Can you work these out from the model? Positions are in its coordinate system, mm. A direction names the side the tool comes from. Give positions to 0.01 mm unless a question says otherwise; leave off trailing zeros. Loops run counter-clockwise (first coordinate to the right, second up) from the corner with the lowest first, then second, coordinate; pieces in that order, holes last. Notation, with made-up numbers: M -5,83 L 20,83 A17 ccw 20,88 Z; hole C 70.5,59 d4. An arc over 180 degrees is marked long. Use CSV: the item, a comma, the result in double quotes.
from build123d import *

# Parameters (mm, degrees)
SKETCH1_R                 = 15
BOSS_EXTRUDE1_DEPTH       = 52
SKETCH2_R                 = 17.5
BOSS_EXTRUDE2_DEPTH       = 43
SKETCH3_R                 = 22.5
BOSS_EXTRUDE3_DEPTH       = 12
SKETCH4_R                 = 15
BOSS_EXTRUDE4_DEPTH       = 40
SKETCH5_R                 = 13.5
BOSS_EXTRUDE5_DEPTH       = 43
SKETCH6_R                 = 12.5
BOSS_EXTRUDE6_DEPTH       = 28
CHAMFER1_SIZE             = 1
CHAMFER2_SIZE             = 1
CHAMFER3_SIZE             = 0.5
CUT_EXTRUDE1_START        = 12.5
CUT_EXTRUDE1_DEPTH        = 20
CUT_EXTRUDE2_START        = 8.5
CUT_EXTRUDE2_DEPTH        = 10
M8X1_0_TAPPED_HOLE1_D     = 7
M8X1_0_TAPPED_HOLE1_DEPTH = 19
M8X1_0_TAPPED_HOLE1_TIP   = 2.103012167


with BuildPart() as part:
    # Sketch1 → Boss-Extrude1 (new body)
    with BuildSketch(Plane.XY):
        with Locations(Location((0, 0, 0), (0, 0, 180))):
            Circle(SKETCH1_R)
    extrude(amount=BOSS_EXTRUDE1_DEPTH)

    # Sketch2 → Boss-Extrude2 (add)
    with BuildSketch(Plane.XY.offset(52)):
        Circle(SKETCH2_R)
    extrude(amount=BOSS_EXTRUDE2_DEPTH)

    # Sketch3 → Boss-Extrude3 (add)
    with BuildSketch(Plane.XY.offset(95)):
        Circle(SKETCH3_R)
    extrude(amount=BOSS_EXTRUDE3_DEPTH)

    # Sketch4 → Boss-Extrude4 (add)
    with BuildSketch(Plane.XY.offset(107)):
        with Locations(Location((0, 0, 0), (0, 0, 180))):
            Circle(SKETCH4_R)
    extrude(amount=BOSS_EXTRUDE4_DEPTH)

    # Sketch5 → Boss-Extrude5 (add)
    with BuildSketch(Plane.XY.offset(147)):
        Circle(SKETCH5_R)
    extrude(amount=BOSS_EXTRUDE5_DEPTH)

    # Sketch6 → Boss-Extrude6 (add)
    with BuildSketch(Plane.XY.offset(190)):
        Circle(SKETCH6_R)
    extrude(amount=BOSS_EXTRUDE6_DEPTH)

    # Chamfer1
    chamfer1_edges = [part.edges().sort_by_distance(p)[0] for p in [
        (15, 0, 0),
    ]]
    chamfer(chamfer1_edges, length=CHAMFER1_SIZE)

    # Chamfer2
    chamfer2_edges = [part.edges().sort_by_distance(p)[0] for p in [
        (15, 0, 147),
        (-12.5, 0, 218),
        (-17.5, 0, 52),
    ]]
    chamfer(chamfer2_edges, length=CHAMFER2_SIZE)

    # Chamfer3
    chamfer3_edges = [part.edges().sort_by_distance(p)[0] for p in [
        (-22.5, 0, 95),
        (-22.5, 0, 107),
    ]]
    chamfer(chamfer3_edges, length=CHAMFER3_SIZE)

    # Sketch7 → Cut-Extrude1 (cut)
    with BuildSketch(Plane(origin=(0, 0, 0), x_dir=(1, 0, 0), z_dir=(0, 1, 0)).offset(CUT_EXTRUDE1_START)):
        with BuildLine():
            Line((5, -67), (5, -82))
            ThreePointArc((5, -82), (0, -87), (-5, -82))
            Line((-5, -82), (-5, -67))
            ThreePointArc((-5, -67), (0, -62), (5, -67))
        make_face()
    extrude(amount=CUT_EXTRUDE1_DEPTH, mode=Mode.SUBTRACT)

    # Sketch8 → Cut-Extrude2 (cut)
    with BuildSketch(Plane(origin=(0, 0, 0), x_dir=(1, 0, 0), z_dir=(0, 1, 0)).offset(CUT_EXTRUDE2_START)):
        with BuildLine():
            Line((4, -198), (4, -210))
            ThreePointArc((4, -210), (0, -214), (-4, -210))
            Line((-4, -210), (-4, -198))
            ThreePointArc((-4, -198), (0, -194), (4, -198))
        make_face()
    extrude(amount=CUT_EXTRUDE2_DEPTH, mode=Mode.SUBTRACT)

    # M8x1.0 Tapped Hole1
    with Locations(Plane.XY.offset(218)):
        with Locations((0, 0)):
            Hole(M8X1_0_TAPPED_HOLE1_D / 2, depth=M8X1_0_TAPPED_HOLE1_DEPTH)
            with Locations((0, 0, -(M8X1_0_TAPPED_HOLE1_DEPTH + M8X1_0_TAPPED_HOLE1_TIP / 2))):  # 118° drill point
                Cone(0, M8X1_0_TAPPED_HOLE1_D / 2, M8X1_0_TAPPED_HOLE1_TIP, mode=Mode.SUBTRACT)


solid = part.part
Q1. If we mould it in two halves opening along Z, with no side actions, what happens to faces 4 (the cylindrical face through (-8.06, -12.65, 26.14)), 5 (the cylindrical face through (0, 15, 87)), 6 (the flat face through (5, 15, 74)), 7 (the flat face through (14.4, 5.2, 107))? For each: released by +Z, released by -Z, zero draft, split by the parting line, or undercut.
Model answer:
face 4,"zero draft"
face 5,"undercut"
face 6,"undercut"
face 7,"released by +Z"
Q2. I want a section at A-A, the plane z = 47. Please give me the cut outline in (x, y).
Model answer:
outline,"C 0,0 d30"
Q3. Please list where these lines run through material, in increasing order: L1, parallel to Y at x = 0, z = 211.5; L2, parallel to X at y = 1, z = 204; L3, parallel to Z at x = 4, y = 14.5. Write a range as from..to.
Model answer:
L1,"-12.5..-3.5, 3.5..8.5"
L2,"-12.46..-3.35, 3.35..12.46"
L3,"52..64, 85..107"
Q4. For faces 1 (the flat face through (0, 8.5, 204)), 2 (the flat face through (-15, -10, 95)), 3 (the cylindrical face through (-3.233, -1.341, 208.367)), which set-ups out of +Z, -Z, +X, -X, +Y, -Y let a thin tool reach every point of the face, with its end or its side?
Model answer:
face 1,"+Y"
face 2,"-Z"
face 3,"+Z"
Q5. I'm going to push flat-ended pins straight in: P1, Ø2, axis at y = 14, z = 76.5, coming from the -X side; P2, Ø4, axis at y = -6, z = 65, coming from the +X side; P3, Ø3, axis at x = 0, z = 78, coming from the +Y side. Where does each tip first touch, or does it pass through?
Model answer:
P1,"x = -11.72"
P2,"x = 17.04"
P3,"y = 12.5"
